Geometry: see drawing. Coordinates: mm, zero at the bounding-box minimum. A direction names the side the tool comes from. Give positions to 0.01 mm unless a question says otherwise; leave off trailing zeros. Order: outer loops, then holes, each group sorted by start corner. A loop starts at its lowest first (then second) coordinate and runs counter-clockwise, first axis right, second up. Notation, with made-up numbers: (71.5, 40) - (115.5, 40) arc R15 ccw to (115.5, 60) - close; hole circle Ø7 at (73, 55). An arc over 180 degrees is marked (long way). One line per question, with ' | ' between items. Start each with the question number.
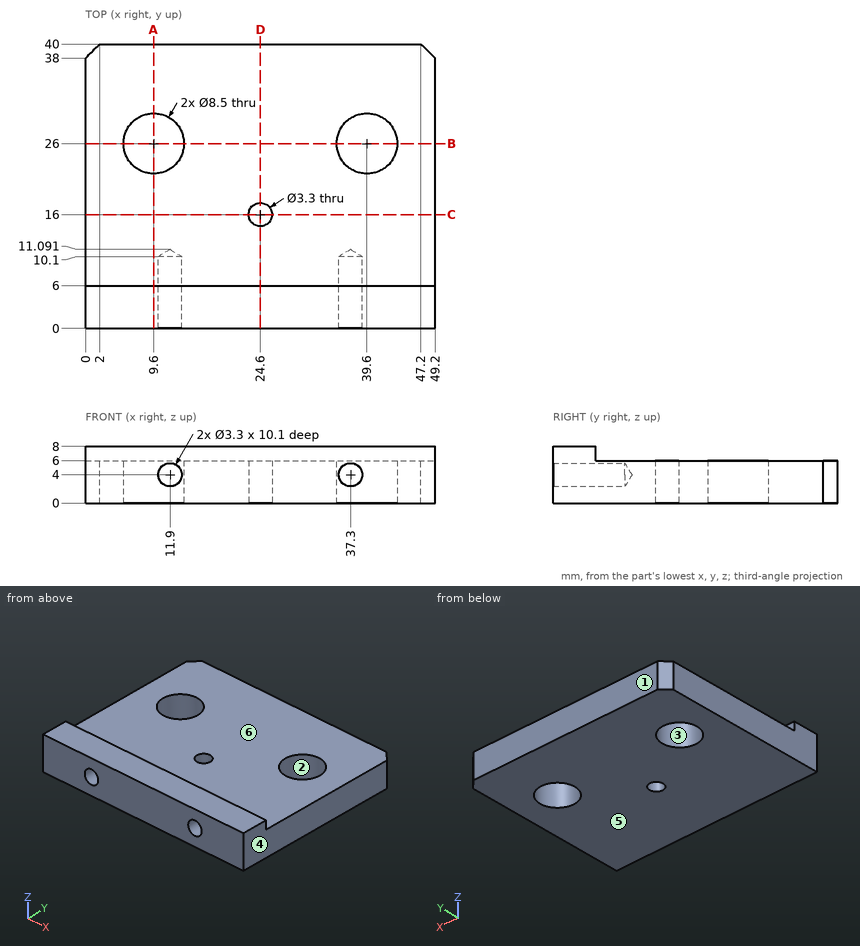
(1) Cut plane B-B, the plane y = 26. Return the cut outline in (x, z), plus the area to 3 significant figures.
(2) Pull-direction query (Y, two-part tool) for the marked faces 1, 2, 3 and 4; classes: +Y half, -Y half, draft (parallel to the pull), parting line (faces both ways), or undercut.
(3) Material intervals for line 1 along X through (y, z) = (3, 4); line 2 along Y through (x, z) = (24.6, 3.55); line 3 along Y through (x, z) = (9.6, 4.1), sorted ascending. Write a range as from..to.
(4) Access query for the marked faces 5 and 6. Directions: +Z, -Z, +X, -X, +Y, -Y. A direction counts if a zero-diameter tool reaches every point of the face in a straight line with its end or side. Return the directions, or none.
(5) Cut plane D-D, the plane x = 24.6. Return the cut outline in (y, z), plus the area to 3 significant figures.
(6) Contact query for flat-ended pins moving along their axis: P1, Ø1.5, axis at x = 32.5, y = 33.5, coming from the +Z side; P2, Ø0.6, axis at x = 34.5, z = 7, coming from the +Y side. Output: stop coordinate, or through.
(7) Cut plane C-C, the plane y = 16. Return the cut outline in (x, z), plus the area to 3 significant figures.
(8) Cut plane A-A, the plane x = 9.6. Return the cut outline in (y, z), plus the area to 3 significant figures.
Results are:
1) outline: (0, 0) - (5.35, 0) - (5.35, 6) - (0, 6) - close; (13.85, 0) - (35.35, 0) - (35.35, 6) - (13.85, 6) - close; (43.85, 0) - (49.2, 0) - (49.2, 6) - (43.85, 6) - close | area: 193 mm2
2) face 1: +Y half | face 2: undercut | face 3: undercut | face 4: draft
3) line 1: 0..10.25, 13.55..35.65, 38.95..49.2 | line 2: 0..14.35, 17.65..40 | line 3: 0..21.75, 30.25..40
4) face 5: -Z, +X, -X, +Y, -Y | face 6: +Z, +X, -X, +Y
5) outline: (0, 0) - (14.35, 0) - (14.35, 6) - (6, 6) - (6, 8) - (0, 8) - close; (17.65, 0) - (40, 0) - (40, 6) - (17.65, 6) - close | area: 232 mm2
6) P1: z = 6 | P2: y = 6
7) outline: (0, 0) - (22.95, 0) - (22.95, 6) - (0, 6) - close; (26.25, 0) - (49.2, 0) - (49.2, 6) - (26.25, 6) - close | area: 275 mm2
8) outline: (0, 0) - (21.75, 0) - (21.75, 6) - (6, 6) - (6, 8) - (0, 8) - close; (30.25, 0) - (40, 0) - (40, 6) - (30.25, 6) - close | area: 201 mm2
